For this review, use the dimensioned drawing (mm, ordinates from the lowest corner) and the shaded views. Give positions to 0.01 mm unless a question says otherwise; leave off trailing zeros. Loops run counter-clockwise (first coordinate to the right, second up) from the corner with the lowest first, then second, coordinate; pieces in that order, holes last. Notation, with made-up numbers: (65, -0.5) - (111, -0.5) arc R16 ccw to (111, 12.5) - close; hole circle Ø9 at (-9.5, -16.5). An arc over 180 degrees is marked (long way). Put each result on its own line as item: value.
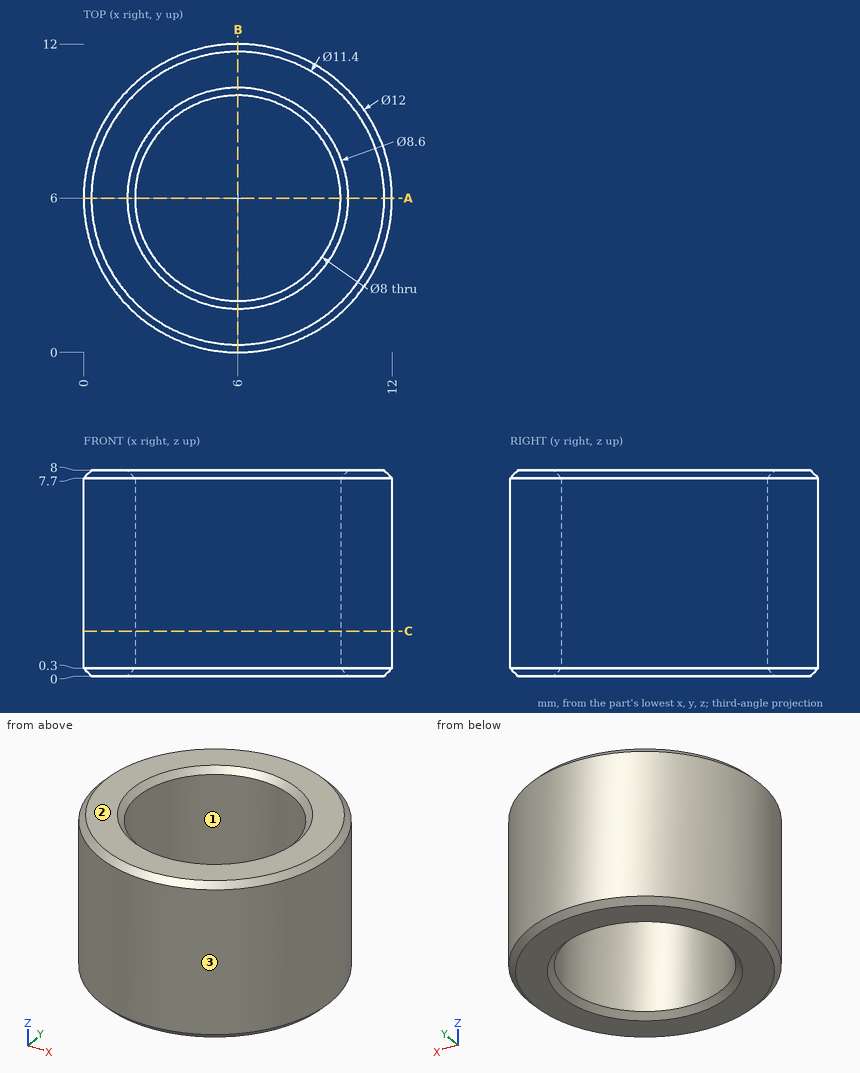
1) Take a section at C-C on z = 1.75. State the section outline as (x, y) points.
Geometry check:
outline: circle Ø12 at (6, 6); hole circle Ø8 at (6, 6)
2) Wall thickness on line 1 (Y direction, x = 6, z = 3.5); line 2 (X direction, y = 9.5, z = 4.75); line 3 (X direction, y = 3.5, z = 5): over which ranges is each line inside the solid? List them lowest first.
Geometry check:
line 1: y = 0 to 2, 10 to 12
line 2: x = 1.13 to 4.06, 7.94 to 10.87
line 3: x = 0.55 to 2.88, 9.12 to 11.45
3) Insertion check: pin 1 Ø1 at (x, y) = (6.5, 8.5) entering from -Z. The pin has a flat end and moves straight along its axis. Give the tip position at first contact, or say it passes through.
Geometry check:
pin 1: passes through
4) Take a section at A-A on y = 6. State the section outline as (x, z) points.
Geometry check:
outline: (0, 0.3) - (0.3, 0) - (1.7, 0) - (2, 0.3) - (2, 7.7) - (1.7, 8) - (0.3, 8) - (0, 7.7) - close; (10, 0.3) - (10.3, 0) - (11.7, 0) - (12, 0.3) - (12, 7.7) - (11.7, 8) - (10.3, 8) - (10, 7.7) - close
5) Draft analysis for pull direction X (two halves, no side actions). For the marked faces 1, 2 and 3, state which applies: pulls with the +X half, pulls with the -X half, needs draft (parallel to the pull), parting line crosses it, or undercut.
Geometry check:
face 1: undercut
face 2: needs draft
face 3: parting line crosses it
